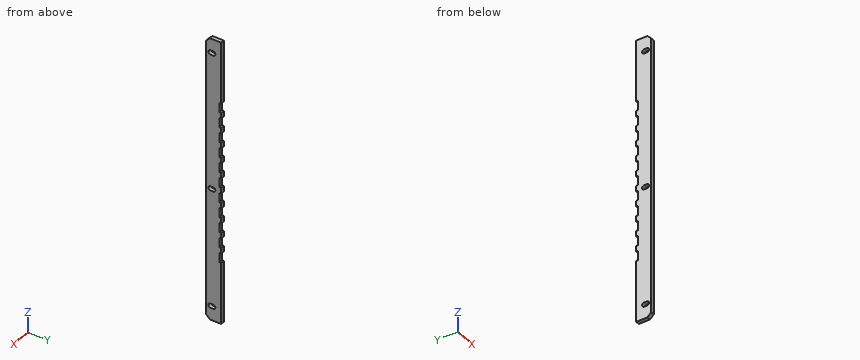
from build123d import *

# Parameters (mm, degrees)
SKETCH_1_W                 = 300
SKETCH_1_H                 = 16
BOSS_EXTRUDE_1_DEPTH       = 4
CHAMFER_1_SIZE             = 4
CUT_EXTRUDE_1_DEPTH        = 151.26643005
SKETCH_3_W                 = 10
SKETCH_3_H                 = 4
CUT_EXTRUDE_2_DEPTH        = 151.26643005
LINEAR_PATTERN_1_COUNT     = 6
LINEAR_PATTERN_1_PITCH     = 16
LINEAR_PATTERN_1_COL_COUNT = 6
LINEAR_PATTERN_1_COL_PITCH = 16
CUT_EXTRUDE_3_DEPTH        = 151.26643005


with BuildPart() as part:
    # Sketch 1 → Boss-Extrude 1 (new body)
    with BuildSketch(Plane(origin=(0, 0, 0), x_dir=(0, 0, -1), z_dir=(1, 0, 0))):
        Rectangle(SKETCH_1_W, SKETCH_1_H)
    extrude(amount=BOSS_EXTRUDE_1_DEPTH)

    # Chamfer 1
    chamfer_1_edges = [part.edges().sort_by_distance(p)[0] for p in [
        (2, -8, -150),
        (2, -8, 150),
    ]]
    chamfer(chamfer_1_edges, length=CHAMFER_1_SIZE)

    # Sketch 2 → Cut-Extrude 1 (cut, through all)
    with BuildSketch(Plane(origin=(4, 0, 0), x_dir=(0, 0, -1), z_dir=(1, 0, 0))):
        with BuildLine():
            Line((-132.75, -0.5), (-132.75, -3.5))
            ThreePointArc((-132.75, -3.5), (-135, -5.75), (-137.25, -3.5))
            Line((-137.25, -3.5), (-137.25, -0.5))
            ThreePointArc((-137.25, -0.5), (-135, 1.75), (-132.75, -0.5))
        make_face()
    cut_extrude_1 = extrude(amount=-CUT_EXTRUDE_1_DEPTH, mode=Mode.SUBTRACT)

    # Mirror 1: Cut-Extrude 1 across plane
    add(cut_extrude_1.mirror(Plane.XY), mode=Mode.SUBTRACT)

    # Sketch 3 → Cut-Extrude 2 (cut, through all)
    with BuildSketch(Plane(origin=(4, 0, 0), x_dir=(0, 0, -1), z_dir=(1, 0, 0))):
        with Locations((0, 8)):
            Rectangle(SKETCH_3_W, SKETCH_3_H)
    cut_extrude_2 = extrude(amount=-CUT_EXTRUDE_2_DEPTH, mode=Mode.SUBTRACT)

    # Linear Pattern 1: Cut-Extrude 2 ×6
    with Locations(*[(0, 0, -i * LINEAR_PATTERN_1_PITCH) for i in range(1, LINEAR_PATTERN_1_COUNT)]):
        add(cut_extrude_2, mode=Mode.SUBTRACT)

    # Linear Pattern 1 col: Cut-Extrude 2 ×6
    with Locations(*[(0, 0, i * LINEAR_PATTERN_1_COL_PITCH) for i in range(1, LINEAR_PATTERN_1_COL_COUNT)]):
        add(cut_extrude_2, mode=Mode.SUBTRACT)

    # Sketch 4 → Cut-Extrude 3 (cut, through all)
    with BuildSketch(Plane(origin=(4, 0, 0), x_dir=(0, 0, -1), z_dir=(1, 0, 0))):
        with BuildLine():
            Line((12.25, -0.5), (12.25, -3.5))
            ThreePointArc((12.25, -3.5), (10, -5.75), (7.75, -3.5))
            Line((7.75, -3.5), (7.75, -0.5))
            ThreePointArc((7.75, -0.5), (10, 1.75), (12.25, -0.5))
        make_face()
    extrude(amount=-CUT_EXTRUDE_3_DEPTH, mode=Mode.SUBTRACT)


solid = part.part
Verification items for the finished model (mm, model axes). Round coordinates to 2 decimals unless told otherwise and drop trailing zeros. Write each question's results on one line, items separated by ' | '.
1) Gauge pin test, flat ends, axial feed: P1, Ø2, axis at x = 2.5, z = 30.5, coming from the +Y side; P2, Ø1, axis at x = 1.5, y = -6, coming from the +Z side. Record the tip position at first contact, or that the pin passes through.
Checks:
P1: stops at y = 6 | P2: stops at z = 148.5
2) Scan lines: L1, parallel to Z at x = 3.5, y = -3; L2, parallel to Z at x = 3.6, y = -4.5; L3, parallel to Y at x = 3.6, z = -17.5. Record each from-to range of solid material in increasing order. Write a range as from..to.
Checks:
L1: z = -150..-137.25, -132.75..-12.25, -7.75..132.75, 137.25..150 | L2: z = -149.5..-137.02, -132.98..-12.02, -7.98..132.98, 137.02..149.5 | L3: y = -8..6
3) Section check A-A on x = 1.9. State how many separate pieces and enclosed holes the cut face has, then the cut area to 3 significant figures.
Checks:
separate pieces: 1 | enclosed holes: 3 | area: 4,480 mm2
